Could you check a few things on this model? Use its own coordinates, in mm. A direction names the side the tool comes from. Give positions to 0.01 mm unless a question says otherwise; leave off trailing zeros. Order: outer loops, then holes, each group sorted by start corner. A loop starts at its lowest first (then second) coordinate and runs counter-clockwise, first axis right, second up. Notation, with made-up numbers: (-16, 20.5) -> (-8, 20.5) arc R13 cw to (-8, 39.5) -> close; hole circle Ø3 at (37, 34). An arc over 180 degrees is marked (long way). Write each question's results on one line, items separated by ' | '.
```python
from build123d import *

# Parameters (mm, degrees)
SKETCH1_R           = 0.75
BOSS_EXTRUDE1_DEPTH = 26
SKETCH2_R           = 1.25
BOSS_EXTRUDE2_DEPTH = 1.5
SKETCH3_OUTSIDE_W   = 10.046
SKETCH3_OUTSIDE_H   = 10.046
SKETCH3_OUTSIDE_R   = 0.6
CUT_EXTRUDE1_DEPTH  = 0.3
CHAMFER1_SIZE       = 0.1


with BuildPart() as part:
    # Sketch1 → Boss-Extrude1 (new body)
    with BuildSketch(Plane(origin=(0, 0, 0), x_dir=(1, 0, 0), z_dir=(0, 1, 0))):
        with Locations(Location((0, 0, 0), (0, 0, 270))):
            Circle(SKETCH1_R)
    extrude(amount=BOSS_EXTRUDE1_DEPTH)

    # Sketch2 → Boss-Extrude2 (add)
    with BuildSketch(Plane(origin=(0, 26, 0), x_dir=(1, 0, 0), z_dir=(0, 1, 0))):
        with Locations(Location((0, 0, 0), (0, 0, 270))):
            Circle(SKETCH2_R)
    extrude(amount=BOSS_EXTRUDE2_DEPTH)

    # Sketch3 outside → Cut-Extrude1 (cut)
    with BuildSketch(Plane(origin=(0, 1, 0), x_dir=(-1, 0, 0), z_dir=(0, -1, 0))):
        Rectangle(SKETCH3_OUTSIDE_W, SKETCH3_OUTSIDE_H)
        with Locations(Location((0, 0, 0), (0, 0, 90))):
            Circle(SKETCH3_OUTSIDE_R, mode=Mode.SUBTRACT)
    extrude(amount=CUT_EXTRUDE1_DEPTH, mode=Mode.SUBTRACT)

    # Chamfer1
    chamfer1_edges = [part.edges().sort_by_distance(p)[0] for p in [
        (0, 0, -0.75),
    ]]
    chamfer(chamfer1_edges, length=CHAMFER1_SIZE)


solid = part.part
```
Q1. For faces 4 (the flat face through (-1, 26, 0)), 5 (the flat face through (0, 0, 0)), which set-ups out of +Z, -Z, +X, -X, +Y, -Y let a thin tool reach every point of the face, with its end or its side?
Here are the results:
face 4: -Y | face 5: +Z, -Z, +X, -X, -Y
Q2. I'm going to push flat-ended pins straight in: pin 1 Ø1 at (y, z) = (17, 0) entering from +X; pin 2 Ø1 at (x, y) = (0.5, 11) entering from -Z. Where does each tip first touch, or does it pass through?
Here are the results:
pin 1: stops at x = 0.75 | pin 2: stops at z = -0.75
Q3. Suppose I cut it at A-A on x = 0. Please give me the cut outline in (y, z), and give its area (4 significant figures).
Here are the results:
outline: (0, -0.65) -> (0.1, -0.75) -> (0.7, -0.75) -> (0.7, -0.6) -> (1, -0.6) -> (1, -0.75) -> (26, -0.75) -> (26, -1.25) -> (27.5, -1.25) -> (27.5, 1.25) -> (26, 1.25) -> (26, 0.75) -> (1, 0.75) -> (1, 0.6) -> (0.7, 0.6) -> (0.7, 0.75) -> (0.1, 0.75) -> (0, 0.65) -> close | area: 42.65 mm²
Q4. I need wall thicknesses on line 1 along Y through (x, z) = (0.2, 1.15); line 2 along Y through (x, z) = (-0.35, -0.6); line 3 along Z through (x, y) = (0.45, 13.5). Which ranges of each line are inside material? Lowest first, please.
Here are the results:
line 1: y = 26 to 27.5 | line 2: y = 0.04 to 0.7, 1 to 27.5 | line 3: z = -0.6 to 0.6
Q5. Thinking about a two-plate mould opening in Y: for faces 1 (the flat face through (0, 27.5, 0)), 2 (the cylindrical face through (-1.22, 26.74, -0.27)), 3 (the cylindrical face through (0.03, 0.85, 0.6)), which applies, +Y half, -Y half, draft (parallel to the pull), parting line (faces both ways), or undercut?
Here are the results:
face 1: +Y half | face 2: draft | face 3: undercut
Q6. Suppose I cut it at D-D on x = -1. Please give me the cut outline in (y, z), and give its area (3 significant figures).
Here are the results:
outline: (26, -0.75) -> (27.5, -0.75) -> (27.5, 0.75) -> (26, 0.75) -> close | area: 2.25 mm²
Q7. Suppose I cut it at B-B on z = 0. Please give me the cut outline in (x, y), and give its area (4 significant figures).
Here are the results:
outline: (-1.25, 26) -> (-0.75, 26) -> (-0.75, 1) -> (-0.6, 1) -> (-0.6, 0.7) -> (-0.75, 0.7) -> (-0.75, 0.1) -> (-0.65, 0) -> (0.65, 0) -> (0.75, 0.1) -> (0.75, 0.7) -> (0.6, 0.7) -> (0.6, 1) -> (0.75, 1) -> (0.75, 26) -> (1.25, 26) -> (1.25, 27.5) -> (-1.25, 27.5) -> close | area: 42.65 mm²
Q8. Suppose I cut it at C-C on y = 11.5. Please give me the cut outline in (x, z), and give its area (3 significant figures).
Here are the results:
outline: circle Ø1.5 at (0, 0) | area: 1.77 mm²
